Here's the drawing with two shaded views (mm, measured from the low corner). I have some questions. Coordinates: 2 decimals unless noted, no trailing zeros. Loops run counter-clockwise (first coordinate to the right, second up) from the corner with the lowest first, then second, coordinate; pieces in that order, holes last. Notation, with made-up numbers: (-11.5, -33) -> (37.5, -33) arc R19 ccw to (37.5, 1) -> close; hole circle Ø1 at (50.25, 27.25). An arc over 180 degrees is marked (long way). Use CSV: the item, a comma, the result in double quotes. Start each with the question number.
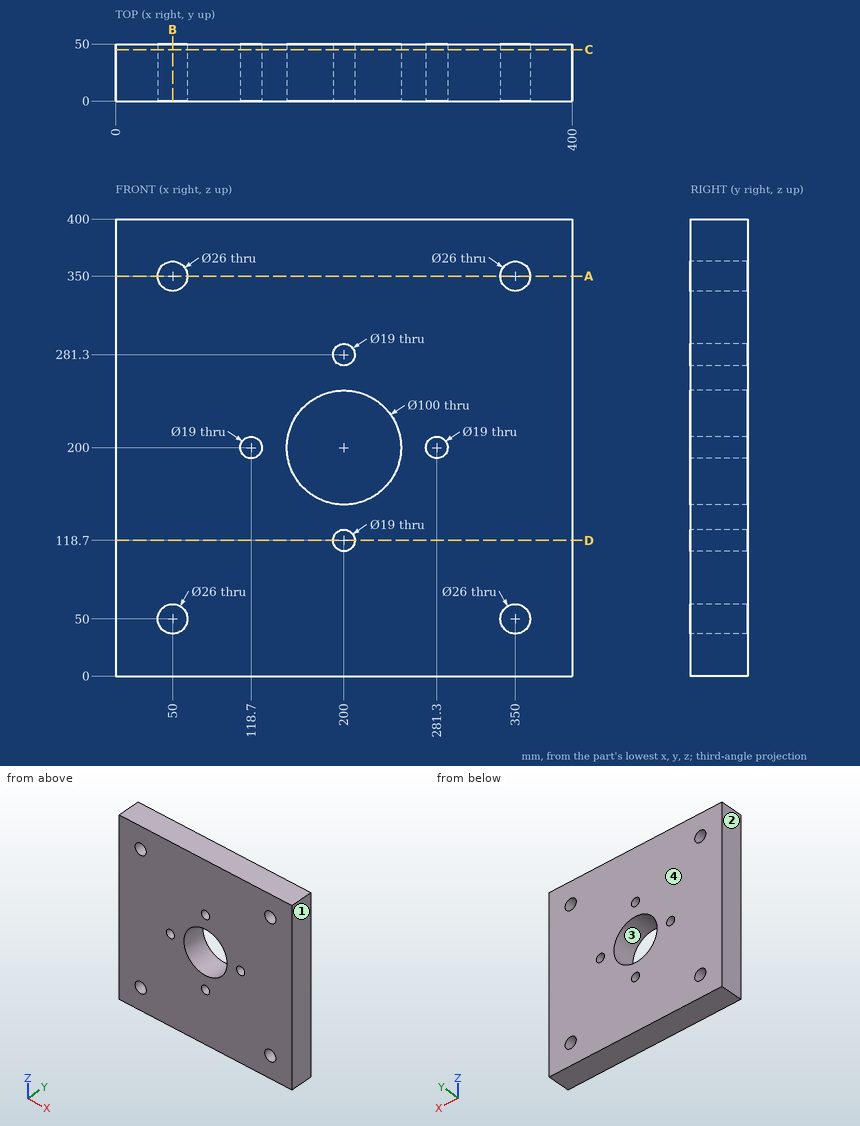
1) I want a section at C-C, the plane y = 45. State how many separate pieces and enclosed holes the cut face has, plus the area to 3 significant figures.
2) I want a section at B-B, the plane x = 50. Please give me the cut outline in (y, z).
3) I want a section at D-D, the plane z = 118.7. Please give me the cut outline in (x, y), plus the area to 4 significant figures.
4) Thinking about a two-plate mould opening in X: for the marked faces 1, 2, 3 and 4, which applies, pulls with the +X half, pulls with the -X half, needs draft (parallel to the pull), parting line crosses it, or undercut?
5) Please list where these lines run through material, in increasing order: L1, parallel to X at y = 36, z = 350; L2, parallel to Z at x = 51.5, y = 34.5; L3, parallel to X at y = 39.5, z = 47. Write a range as [from, to].
6) For P1, Ø2, axis at y = 34.5, z = 133, coming from the -X side, with a flat end and sliding along its axis, tell me the tip position at first contact or that it passes through.
7) I want a section at A-A, the plane z = 350. Please give me the cut outline in (x, y).
Return value:
1,separate pieces,"1"
1,enclosed holes,"9"
1,area,"149,000 mm²"
2,outline,"(0, 0) -> (50, 0) -> (50, 37) -> (0, 37) -> close; (0, 63) -> (50, 63) -> (50, 337) -> (0, 337) -> close; (0, 363) -> (50, 363) -> (50, 400) -> (0, 400) -> close"
3,outline,"(0, 0) -> (190.5, 0) -> (190.5, 50) -> (0, 50) -> close; (209.5, 0) -> (400, 0) -> (400, 50) -> (209.5, 50) -> close"
3,area,"19,050 mm²"
4,face 1,"pulls with the +X half"
4,face 2,"pulls with the -X half"
4,face 3,"undercut"
4,face 4,"needs draft"
5,L1,"x = [0, 37], [63, 337], [363, 400]"
5,L2,"z = [0, 37.09], [62.91, 337.09], [362.91, 400]"
5,L3,"x = [0, 37.35], [62.65, 337.35], [362.65, 400]"
6,P1,"stops at x = 0"
7,outline,"(0, 0) -> (37, 0) -> (37, 50) -> (0, 50) -> close; (63, 0) -> (337, 0) -> (337, 50) -> (63, 50) -> close; (363, 0) -> (400, 0) -> (400, 50) -> (363, 50) -> close"
